Can you work these out from the model? Positions are in its coordinate system, mm. Face numbers are marked on the shaded views. Give positions to 0.01 mm unless a question says otherwise; leave off trailing zeros. Write each loop counter-clockwise with the first axis right and the second up, starting at its lowest first coordinate (ties: lowest second). Pieces come first, ordered by that corner, then holes. Notation, with made-up numbers: M -9,65.25 L 23,65.25 A34 ccw 23,104.25 Z; hole C -5,46.25 d10. An arc over 180 degrees is marked long. Write each question's results on one line, items separated by ' | '.
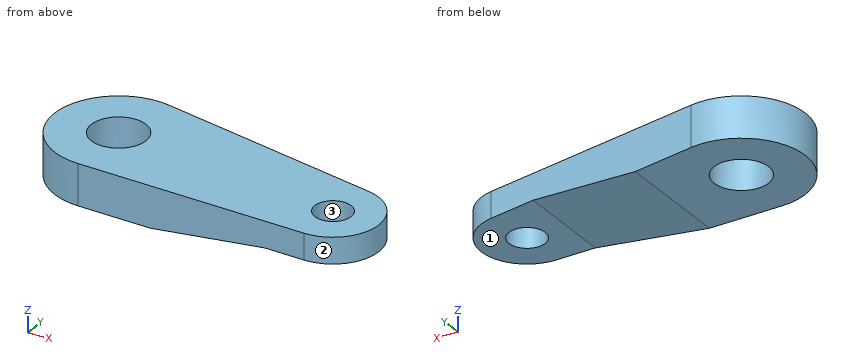
from build123d import *

# Parameters (mm, degrees)
SKETCH1_R               = 2
SKETCH1_R_2             = 3
BOSS_EXTRUDE1_DEPTH     = 6
CUT_EXTRUDE1_DEPTH      = 27.36555884
CUT_EXTRUDE1_DEPTH_BACK = 27.36555884


with BuildPart() as part:
    # Sketch1 → Boss-Extrude1 (new body)
    with BuildSketch(Plane.XY):
        with BuildLine():
            Line((-7.993562913, -0.787462727), (16.925257698, -0.787462727))
            ThreePointArc((16.925257698, -0.787462727), (21.941546469, 3.839929946), (17.733101807, 9.212537273))
            Line((17.733101807, 9.212537273), (-6.862581161, 13.212537273))
            ThreePointArc((-6.862581161, 13.212537273), (-15.016367191, 6.825553227), (-7.993562913, -0.787462727))
        make_face()
        with Locations((16.925257698, 4.245167879)):
            Circle(SKETCH1_R, mode=Mode.SUBTRACT)
        with Locations((-7.993562913, 6.258220121)):
            Circle(SKETCH1_R_2, mode=Mode.SUBTRACT)
    extrude(amount=BOSS_EXTRUDE1_DEPTH)

    # Sketch2 → Cut-Extrude1 (cut, two sides: drawn at the far end of the back side and taken through both)
    with BuildSketch(Plane(origin=(0, 0, 0), x_dir=(1, 0, 0), z_dir=(0, 1, 0)).offset(-CUT_EXTRUDE1_DEPTH_BACK)):
        Polygon((29.386629895, -3.141643917), (12.58106894, -3.141643917), (0, -1.491733663), (-17.019149761, -1.491733663), (-15.478750308, 10.25428202), (32.017830731, 8.260226372), align=None)
    extrude(amount=CUT_EXTRUDE1_DEPTH + CUT_EXTRUDE1_DEPTH_BACK, mode=Mode.SUBTRACT)


solid = part.part
Item 1: I'm going to push flat-ended pins straight in: pin 1 (5 mm diameter, centred on x = -7.99, y = 6.26, fed in from +Z); pin 2 (4.5 mm diameter, centred on x = 19, y = 3.5, fed in from -Z). Where does each tip first touch, or does it pass through?
Geometry says:
pin 1: passes through | pin 2: stops at z = 3.14
Item 2: If I drill on line 1 (X direction, y = 4.75, z = 3.95); line 2 (Y direction, x = -6, z = 2.5); line 3 (X direction, y = 7.5, z = 3.45), over which ranges is the centre line in solid material (lowest first)? Write a range as from..to.
Geometry says:
line 1: x = -14.88..-10.59, -5.4..14.99, 18.86..21.93 | line 2: y = -0.79..4.02, 8.5..13.07 | line 3: x = -14.93..-10.72, -5.26..20.76
Item 3: Thinking about a two-plate mould opening in X: for the marked faces 1, 2 and 3, which applies, +X half, -X half, draft (parallel to the pull), parting line (faces both ways), or undercut?
Geometry says:
face 1: draft | face 2: +X half | face 3: undercut
Item 4: I want a section at B-B, the plane x = -9.5. Please give me the cut outline in (y, z).
Geometry says:
outline: M -0.62,1.49 L 3.66,1.49 L 3.66,6 L -0.62,6 Z; M 8.85,1.49 L 13.14,1.49 L 13.14,6 L 8.85,6 Z
Item 5: I want a section at C-C, the plane z = 2.2. Please give me the cut outline in (x, y).
Geometry says:
outline: M -7.99,-0.79 L 5.4,-0.79 L 5.4,11.22 L -6.86,13.21 A7.05 ccw long Z; hole C -7.99,6.26 d6
Item 6: I want a section at A-A, the plane y = 8.75. Please give me the cut outline in (x, z).
Geometry says:
outline: M -14.58,1.49 L -9.66,1.49 L -9.66,6 L -14.58,6 Z; M -6.32,1.49 L 0,1.49 L 12.58,3.14 L 19.17,3.14 L 19.17,6 L -6.32,6 Z
Item 7: I want a section at D-D, the plane z = 3.65. Please give me the cut outline in (x, y).
Geometry says:
outline: M -7.99,-0.79 L 16.93,-0.79 A5.03 ccw 17.73,9.21 L -6.86,13.21 A7.05 ccw long Z; hole C -7.99,6.26 d6; hole C 16.93,4.25 d4
